The listing builds one solid part. Answer for the finished solid, in the listing's coordinates (mm). A direction names the side the tool comes from. Coordinates: 2 decimals unless noted, no trailing zeros. Loops run counter-clockwise (first coordinate to the right, second up) from the corner with the lowest first, then second, coordinate; pieces in that order, holes last. Notation, with made-up numbers: (76, 77) - (117, 77) arc R29 ccw to (117, 106) - close; hole circle Ø9 at (24.5, 67.25). An arc over 180 degrees is marked (long way). Put each result on its own line as item: value.
```python
from build123d import *

# Parameters (mm, degrees)
EXTRUDE_1_DEPTH           = 4
SKETCH_2_W                = 4
SKETCH_2_H                = 80
EXTRUDE_2_DEPTH           = 41
CUT_EXTRUDE_1_DEPTH       = 140.749776386
CUT_EXTRUDE_2_DEPTH       = 137.711374801
HOLE_WIZARD_18_5_18_5_1_D = 18.5
CHAMFER_1_SIZE            = 5
CHAMFER_2_SIZE            = 30.886890423
FILLET_1_R                = 4
FILLET_2_R                = 8


with BuildPart() as part:
    # 草图1 → 凸台-拉伸1 (new body)
    with BuildSketch(Plane(origin=(0, 0, 0), x_dir=(0, 0, -1), z_dir=(1, 0, 0))):
        Polygon((-45, 0), (27, 40), (-45, 80), (-80, 80), (-80, 0), align=None)
    extrude(amount=-EXTRUDE_1_DEPTH)

    # 草图2 → 凸台-拉伸2 (add)
    with BuildSketch(Plane(origin=(0, 0, 0), x_dir=(0, 0, -1), z_dir=(1, 0, 0))):
        with Locations((-78, 40)):
            Rectangle(SKETCH_2_W, SKETCH_2_H)
    extrude(amount=EXTRUDE_2_DEPTH)

    # 草图3 → 切除-拉伸1 (cut, through all)
    with BuildSketch(Plane.XY.offset(80)):
        with BuildLine():
            Line((34.5, 61), (34.5, 69))
            ThreePointArc((34.5, 69), (31, 72.5), (27.5, 69))
            Line((27.5, 69), (27.5, 61))
            ThreePointArc((27.5, 61), (31, 57.5), (34.5, 61))
        make_face()
    extrude(amount=-CUT_EXTRUDE_1_DEPTH, mode=Mode.SUBTRACT)

    # 草图4 → 切除-拉伸2 (cut, through all)
    with BuildSketch(Plane(origin=(0, 0, 76), x_dir=(-1, 0, 0), z_dir=(0, 0, -1))):
        with BuildLine():
            Line((-34.5, 19), (-34.5, 11))
            ThreePointArc((-34.5, 11), (-31, 7.5), (-27.5, 11))
            Line((-27.5, 11), (-27.5, 19))
            ThreePointArc((-27.5, 19), (-31, 22.5), (-34.5, 19))
        make_face()
    extrude(amount=-CUT_EXTRUDE_2_DEPTH, mode=Mode.SUBTRACT)

    # Ø18.5 (18.5) 直径孔1 (through all)
    with Locations(Plane(origin=(0, 0, 0), x_dir=(0, 0, -1), z_dir=(1, 0, 0))):
        with Locations((-15, 40)):
            Hole(HOLE_WIZARD_18_5_18_5_1_D / 2)

    # 倒角1
    chamfer_1_edges = [part.edges().sort_by_distance(p)[0] for p in [
        (41, 0, 78),
        (41, 80, 78),
    ]]
    chamfer(chamfer_1_edges, length=CHAMFER_1_SIZE)

    # 倒角2
    chamfer_2_edges = [part.edges().sort_by_distance(p)[0] for p in [
        (-2, 40, -27),
    ]]
    chamfer(chamfer_2_edges, length=CHAMFER_2_SIZE)

    # 圆角1
    fillet_1_edges = [part.edges().sort_by_distance(p)[0] for p in [
        (0, 40, 76),
    ]]
    fillet(fillet_1_edges, radius=FILLET_1_R)

    # 圆角2
    fillet_2_edges = [part.edges().sort_by_distance(p)[0] for p in [
        (-4, 40, 80),
    ]]
    fillet(fillet_2_edges, radius=FILLET_2_R)


solid = part.part
```
1) For faces 1 (the face through (38, 78, 78)), 2 (the face through (27.5, 65, 78)), 3 (the face through (22, 39, 76)), determine the directions among +Z, -Z, +X, -X, +Y, -Y from which every point of the face is accessible in a straight line to the end or side of a thin tool.
Found:
face 1: +Z, -Z, +X, +Y
face 2: +Z, -Z
face 3: -Z, +X, +Y, -Y
2) For a pull along Y with two mould halves and no side action, classify faces 4 (the face through (31.1, 72.5, 78)), 5 (the face through (-2, 40, 0)), 6 (the face through (-1.97, 67.33, 22.19)), 7 (the face through (8, 0, 77)) as pulls with the +Y half, pulls with the -Y half, needs draft (parallel to the pull), parting line crosses it, or undercut.
Found:
face 4: undercut
face 5: needs draft
face 6: pulls with the +Y half
face 7: pulls with the -Y half
3) The part is cut by section A-A (x = 31). Give the vertices of the cut face in (y, z).
Found:
outline: (0, 76) - (7.5, 76) - (7.5, 80) - (0, 80) - close; (22.5, 76) - (57.5, 76) - (57.5, 80) - (22.5, 80) - close; (72.5, 76) - (80, 76) - (80, 80) - (72.5, 80) - close
4) Each of these flat-tipped pins is pushed along its axis until it touches: pin 1 (8 mm diameter, centred on x = 29, y = 64, fed in from -Z); pin 2 (2 mm diameter, centred on y = 16.5, z = 78.5, fed in from -X); pin 3 (3 mm diameter, centred on y = 44.5, z = 44.5, fed in from +X). Where does it stop, or does it pass through?
Found:
pin 1: stops at z = 76
pin 2: stops at x = -1.81
pin 3: stops at x = 0
5) Straight lines are drawn through the part: L1, parallel to X at y = 48.5, z = 7; L2, parallel to Y at x = -1, z = 15; L3, parallel to Z at x = 34.5, y = 22. For each, find the intervals that lie inside material, in ascending order. Write a range as [from, to].
Found:
L1: x = [-4, 0]
L2: y = [16.67, 30.75], [49.25, 63.33]
L3: z = [76, 80]
6) The part is cut by section C-C (y = 47). Give the vertices of the cut face in (x, z).
Found:
outline: (-4, 0) - (0, 0) - (0, 8.95) - (-4, 8.95) - close; (-4, 21.05) - (0, 21.05) - (0, 72) arc R4 cw to (4, 76) - (41, 76) - (41, 80) - (4, 80) arc R8 ccw to (-4, 72) - close
7) The part is cut by section B-B (z = 21). Give the vertices of the cut face in (x, y), and give its area (3 significant figures).
Found:
outline: (-4, 13.33) - (0, 13.33) - (0, 32.96) - (-4, 32.96) - close; (-4, 47.04) - (0, 47.04) - (0, 66.67) - (-4, 66.67) - close
area: 157 mm^2
8) The part is cut by section D-D (z = 48). Give the vertices of the cut face in (x, y), and give its area (3 significant figures).
Found:
outline: (-4, 0) - (0, 0) - (0, 80) - (-4, 80) - close
area: 320 mm^2
